from build123d import *

# Parameters (mm, degrees)
SKETCH1_R             = 82.5
SKETCH1_R_2           = 60
BOSS_EXTRUDE1_DEPTH   = 10
SKETCH2_R             = 78
SKETCH2_R_2           = 60
BOSS_EXTRUDE2_DEPTH   = 5
CHAMFER1_SIZE         = 1
M8_TAPPED_HOLE1_D     = 6.8
M8_TAPPED_HOLE1_DEPTH = 12
M8_TAPPED_HOLE1_TIP   = 2.042926105


with BuildPart() as part:
    # Sketch1 → Boss-Extrude1 (new body)
    with BuildSketch(Plane.XY):
        Circle(SKETCH1_R)
        Circle(SKETCH1_R_2, mode=Mode.SUBTRACT)
    extrude(amount=BOSS_EXTRUDE1_DEPTH)

    # Sketch2 → Boss-Extrude2 (add)
    with BuildSketch(Plane.XY.offset(10)):
        Circle(SKETCH2_R)
        Circle(SKETCH2_R_2, mode=Mode.SUBTRACT)
    extrude(amount=BOSS_EXTRUDE2_DEPTH)

    # Chamfer1
    chamfer1_edges = [part.edges().sort_by_distance(p)[0] for p in [
        (-78, 0, 15),
        (-82.5, 0, 0),
    ]]
    chamfer(chamfer1_edges, length=CHAMFER1_SIZE)

    # M8 Tapped Hole1
    with Locations(Plane(origin=(35, 60.621778265, 0), x_dir=(-1, 0, 0), z_dir=(0, 0, -1))):
        with Locations((0, 0), (70, 0), (105, -60.621778265), (70, -121.24355653), (0, -121.24355653), (-35, -60.621778265)):
            Hole(M8_TAPPED_HOLE1_D / 2, depth=M8_TAPPED_HOLE1_DEPTH)
            with Locations((0, 0, -(M8_TAPPED_HOLE1_DEPTH + M8_TAPPED_HOLE1_TIP / 2))):  # 118° drill point
                Cone(0, M8_TAPPED_HOLE1_D / 2, M8_TAPPED_HOLE1_TIP, mode=Mode.SUBTRACT)


solid = part.part
Model file for the job. Use its own axes, mm. A direction names the side the tool comes from. Give positions to 0.01 mm unless a question says otherwise; leave off trailing zeros. Order: outer loops, then holes, each group sorted by start corner. A loop starts at its lowest first (then second) coordinate and runs counter-clockwise, first axis right, second up. Notation, with made-up numbers: (85, -28.5) - (128, -28.5) arc R19 ccw to (128, -20.5) - close; hole circle Ø7 at (75.25, 7.5). An arc over 180 degrees is marked (long way). Write item = value, one per line. Start each with the question number.
1. Drop flat-ended pins along their axis: P1, Ø6, axis at x = 35, y = -60.62, coming from the -Z side; P2, Ø4, axis at y = -35.5, z = 13, coming from the -X side; P3, Ø12, axis at x = -34.5, y = 36.5, coming from the -Z side; P4, Ø5, axis at x = -63.5, z = 11, coming from the -Y side. Give the stop position or say it passes through.
2. Probe line 1 along Y through (x, z) = (0, 4); line 2 along Y through (x, z) = (35, 5.75); line 3 along X through (y, z) = (8, 2.25). List the from-to ranges inside material, lowest first.
3. Cut at B-B, the plane z = 3. List the corners of the cut face in (x, y).
4. Which spindle directions (+Z, -Z, +X, -X, +Y, -Y) get a long thin tool onto all of the face, cutting with end or side? Do faces 1 (the cylindrical face through (-72.698, -2.069, 6.084)), 2 (the flat face through (-43, 43, 0)), 3 (the flat face through (61, 49, 10)). Say none if no direction does.
5. Cut at A-A, the plane x = 0. List the corners of the cut face in (y, z), and give its area (3 significant figures).
6. Two-plate mould, pull along X, no slides. Class faces 4 (the conical face through (34.728, -61.146, 13.688)), 5 (the flat face through (45, -40, 15)), 6 (the cylindrical face through (-17.88, -80.54, 5.44)), 7 (the cylindrical face through (-59.94, 2.64, 7.4)): pulls with the +X half, pulls with the -X half, needs draft (parallel to the pull), parting line crosses it, or undercut.
Taken from the geometry:
q1.P1 = 12.24
q1.P2 = -70.44
q1.P3 = through
q1.P4 = -55.31
q2.line_1 = -82.5 to -60, 60 to 82.5
q2.line_2 = -74.71 to -64.02, -57.22 to -48.73, 48.73 to 57.22, 64.02 to 74.71
q2.line_3 = -82.11 to -59.46, 59.46 to 82.11
q3.outline = circle Ø165 at (0, 0); hole circle Ø6.8 at (-70, 0); hole circle Ø120 at (0, 0); hole circle Ø6.8 at (-35, -60.62); hole circle Ø6.8 at (-35, 60.62); hole circle Ø6.8 at (35, -60.62); hole circle Ø6.8 at (35, 60.62); hole circle Ø6.8 at (70, 0)
q4.face_1 = -Z
q4.face_2 = -Z, +X, -X, +Y, -Y
q4.face_3 = +Z
q5.outline = (-82.5, 1) - (-81.5, 0) - (-60, 0) - (-60, 15) - (-77, 15) - (-78, 14) - (-78, 10) - (-82.5, 10) - close; (60, 0) - (81.5, 0) - (82.5, 1) - (82.5, 10) - (78, 10) - (78, 14) - (77, 15) - (60, 15) - close
q5.area = 628 mm²
q6.face_4 = undercut
q6.face_5 = needs draft
q6.face_6 = parting line crosses it
q6.face_7 = undercut
